Can you work these out from the drawing? Everything is in mm from the part's minimum corner. A direction names the side the tool comes from. Give positions to 0.01 mm unless a question says otherwise; leave off trailing zeros. Loops run counter-clockwise (first coordinate to the right, second up) from the corner with the lowest first, then second, coordinate; pieces in that order, holes last. Notation, with made-up numbers: M 38.5,60.5 L 68.5,60.5 A30 cw 68.5,91.5 Z; hole C -25,39.5 d8. An arc over 180 degrees is marked long. Use CSV: the item, a comma, the result in double quotes.
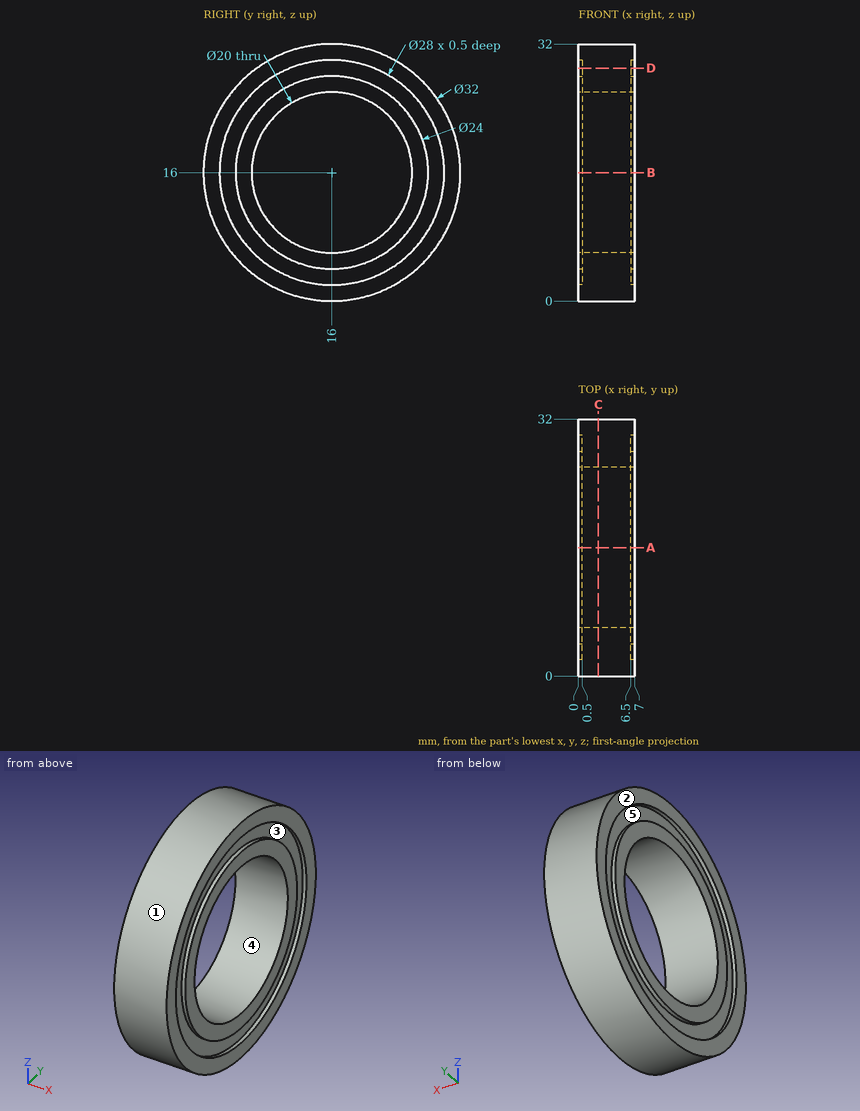
Q1. If we mould it in two halves opening along Z, with no side actions, what happens to the marked faces 1, 2 and 3? For each: released by +Z, released by -Z, zero draft, split by the parting line, or undercut.
Model answer:
face 1,"split by the parting line"
face 2,"zero draft"
face 3,"undercut"
Q2. I want a section at C-C, the plane x = 2.5. Please give me the cut outline in (y, z), then the cut area to 3 significant figures.
Model answer:
outline,"C 16,16 d32; hole C 16,16 d20"
area,"490 mm2"
Q3. I want a section at A-A, the plane y = 16. Please give me the cut outline in (x, z).
Model answer:
outline,"M 0,0 L 7,0 L 7,2 L 6.5,2 L 6.5,4 L 7,4 L 7,6 L 0,6 L 0,4 L 0.5,4 L 0.5,2 L 0,2 Z; M 0,26 L 7,26 L 7,28 L 6.5,28 L 6.5,30 L 7,30 L 7,32 L 0,32 L 0,30 L 0.5,30 L 0.5,28 L 0,28 Z"
Q4. Please list where these lines run through material, in increasing order: L1, parallel to Y at x = 6.95, z = 16; L2, parallel to Z at x = 3, y = 16. Write a range as from..to.
Model answer:
L1,"0..2, 4..6, 26..28, 30..32"
L2,"0..6, 26..32"
Q5. For the marked faces 4 and 5, which set-ups out of +Z, -Z, +X, -X, +Y, -Y let a thin tool reach every point of the face, with its end or its side?
Model answer:
face 4,"+X, -X"
face 5,"-X"
Q6. I want a section at D-D, the plane z = 29. Please give me the cut outline in (x, y), then the cut area to 3 significant figures.
Model answer:
outline,"M 0,6.67 L 7,6.67 L 7,10.8 L 6.5,10.8 L 6.5,21.2 L 7,21.2 L 7,25.33 L 0,25.33 L 0,21.2 L 0.5,21.2 L 0.5,10.8 L 0,10.8 Z"
area,"120 mm2"
Q7. I'm going to push flat-ended pins straight in: P1, Ø1, axis at x = 5.5, y = 20.5, coming from the -Z side; P2, Ø1, axis at x = 2.5, z = 27.5, coming from the +Y side; P3, Ø17, axis at y = 16, z = 16, coming from the -X side; P4, Ø2, axis at x = 2, y = 12.5, coming from the +Z side. Where does each tip first touch, or does it pass through?
Model answer:
P1,"z = 0.51"
P2,"y = 27.62"
P3,"through"
P4,"z = 31.8"
